from build123d import *

# Parameters (mm, degrees)
SKETCH1_W           = 130
SKETCH1_H           = 130
BOSS_EXTRUDE1_DEPTH = 10
SKETCH2_R           = 42.5
BOSS_EXTRUDE2_DEPTH = 5
SKETCH3_R           = 5
CUT_EXTRUDE1_DEPTH  = 51


with BuildPart() as part:
    # Sketch1 → Boss-Extrude1 (new body)
    with BuildSketch(Plane.XY):
        Rectangle(SKETCH1_W, SKETCH1_H)
    extrude(amount=BOSS_EXTRUDE1_DEPTH)

    # Sketch2 → Boss-Extrude2 (add)
    with BuildSketch(Plane.XY.offset(10)):
        Circle(SKETCH2_R)
    extrude(amount=BOSS_EXTRUDE2_DEPTH)

    # Sketch3 → Cut-Extrude1 (cut)
    with BuildSketch(Plane.XY.offset(10)):
        with Locations((50, 50)):
            Circle(SKETCH3_R)
        with Locations((-50, 50)):
            Circle(SKETCH3_R)
        with Locations((-50, -50)):
            Circle(SKETCH3_R)
        with Locations((50, -50)):
            Circle(SKETCH3_R)
    extrude(amount=-CUT_EXTRUDE1_DEPTH, mode=Mode.SUBTRACT)


solid = part.part
Input: part model. Units: mm. Frame: model coordinates. A direction names the side the tool comes from. Coordinates: 2 decimals unless noted, no trailing zeros. Loops run counter-clockwise (first coordinate to the right, second up) from the corner with the lowest first, then second, coordinate; pieces in that order, holes last. Notation, with made-up numbers: (-21.5, 42.25) - (-12.5, 42.25) arc R34 cw to (-12.5, 79.25) - close; hole circle Ø11 at (-16, -39). An arc over 180 degrees is marked (long way). Answer in a Markdown table with one row per item. Add a question column.
Item 1: Mould query, pull axis Y, two halves, no side actions, for faces 1 (the cylindrical face through (-54, -47, 5)), 2 (the flat face through (-1, 65, 5)), 3 (the flat face through (-1, 1, 15)). Classes: released by +Y, released by -Y, zero draft, split by the parting line, or undercut.
Item 2: Contact query for flat-ended pins moving along their axis: P1, Ø9, axis at x = 50, y = -50, coming from the -Z side; P2, Ø3, axis at x = 19.5, z = 12.5, coming from the -Y side; P3, Ø3, axis at y = 1.5, z = 13, coming from the +X side. Output: stop coordinate, or through.
Item 3: Line query: line 1 along Y through (x, z) = (50, 3.5); line 2 along X through (y, z) = (48, 6.5); line 3 along Z through (x, y) = (-39, 26). Output: solid intervals per line, ascending. Write a range as [from, to].
Item 4: Section query C-C on z = 7.5. Return the cut outline in (x, y).
Item 5: Section query A-A on x = -50. Return the cut outline in (y, z), then the cut area to 3 significant figures.
Item 6: Section query D-D on y = 0. Return the cut outline in (x, z).
Item 7: Access query for faces 4 (the cylindrical face through (49.349, 54.957, 5.07)), 5 (the flat face through (-44, 1, 10)). Directions: +Z, -Z, +X, -X, +Y, -Y. A direction counts if a zero-diameter tool reaches every point of the face in a straight line with its end or side. Return the directions, or none.
Recorded:
| question | item | result |
|---|---|---|
| 1 | face 1 | undercut |
| 1 | face 2 | released by +Y |
| 1 | face 3 | zero draft |
| 2 | P1 | through |
| 2 | P2 | y = -38.5 |
| 2 | P3 | x = 42.5 |
| 3 | line 1 | [-65, -55], [-45, 45], [55, 65] |
| 3 | line 2 | [-65, -54.58], [-45.42, 45.42], [54.58, 65] |
| 3 | line 3 | [0, 10] |
| 4 | outline | (-65, -65) - (65, -65) - (65, 65) - (-65, 65) - close; hole circle Ø10 at (-50, -50); hole circle Ø10 at (-50, 50); hole circle Ø10 at (50, -50); hole circle Ø10 at (50, 50) |
| 5 | outline | (-65, 0) - (-55, 0) - (-55, 10) - (-65, 10) - close; (-45, 0) - (45, 0) - (45, 10) - (-45, 10) - close; (55, 0) - (65, 0) - (65, 10) - (55, 10) - close |
| 5 | area | 1,100 mm^2 |
| 6 | outline | (-65, 0) - (65, 0) - (65, 10) - (42.5, 10) - (42.5, 15) - (-42.5, 15) - (-42.5, 10) - (-65, 10) - close |
| 7 | face 4 | +Z, -Z |
| 7 | face 5 | +Z |
